Here's the drawing with two shaded views (mm, measured from the low corner). I have some questions. A direction names the side the tool comes from. Round coordinates to 2 decimals unless told otherwise and drop trailing zeros. Loops run counter-clockwise (first coordinate to the right, second up) from the corner with the lowest first, then second, coordinate; pieces in that order, holes last.
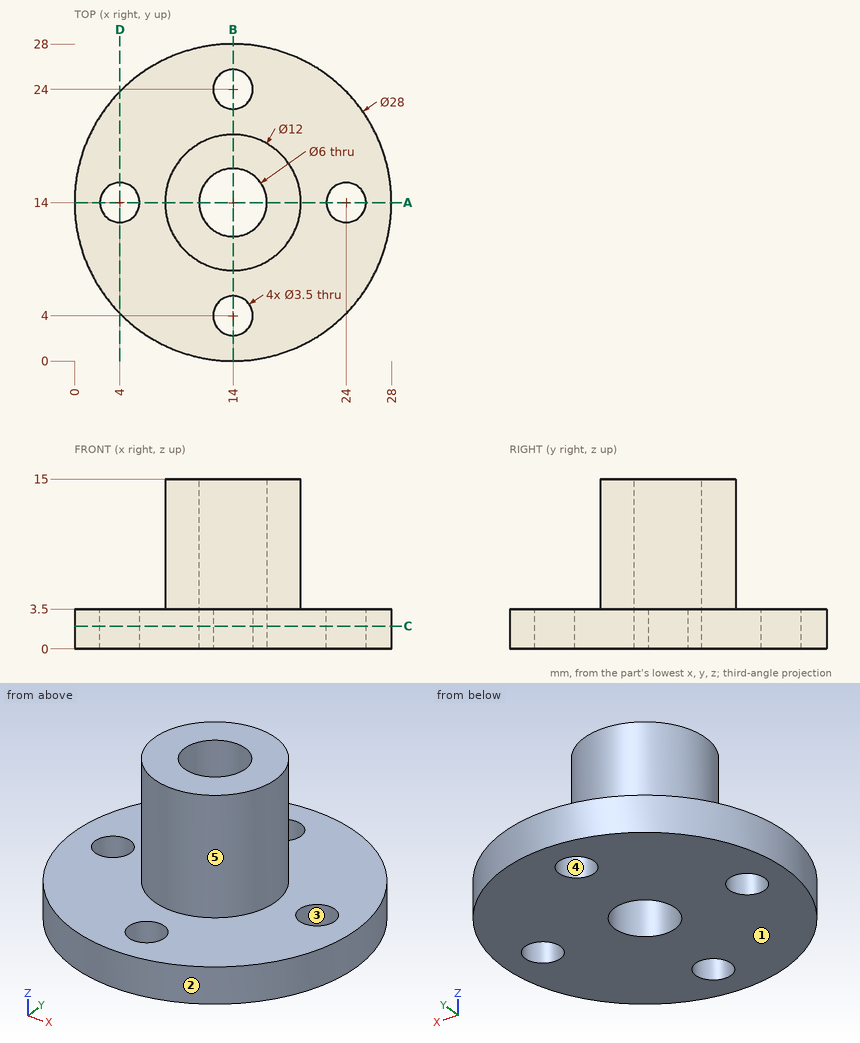
Item 1: Will these pins go through, and if not, where does the flat tip stop? pin 1 (5.5 mm diameter, centred on x = 14, y = 24, fed in from +Z); pin 2 (5 mm diameter, centred on x = 9.5, z = 5.5, fed in from -Y); pin 3 (1.5 mm diameter, centred on x = 11.5, z = 12.5, fed in from -Y).
Results list:
pin 1: stops at z = 3.5
pin 2: stops at y = 0.33
pin 3: stops at y = 8.26
Item 2: If we section it at A-A, the plane y = 14: Please give me the cut outline in (x, z).
Results list:
outline: (0, 0) - (2.25, 0) - (2.25, 3.5) - (0, 3.5) - close; (5.75, 0) - (11, 0) - (11, 15) - (8, 15) - (8, 3.5) - (5.75, 3.5) - close; (17, 0) - (22.25, 0) - (22.25, 3.5) - (20, 3.5) - (20, 15) - (17, 15) - close; (25.75, 0) - (28, 0) - (28, 3.5) - (25.75, 3.5) - close
Item 3: If I drill on line 1 along Y through (x, z) = (14, 2.7); line 2 along Y through (x, z) = (14, 11.25); line 3 along Z through (x, y) = (6, 22.75), over which ranges is the centre line in solid material (lowest first)?
Results list:
line 1: y = 0 to 2.25, 5.75 to 11, 17 to 22.25, 25.75 to 28
line 2: y = 8 to 11, 17 to 20
line 3: z = 0 to 3.5
Item 4: We'd pull the mould along X, two halves only. Please class the marked faces 1, 2 and 3: released by +X, released by -X, zero draft, split by the parting line, or undercut.
Results list:
face 1: zero draft
face 2: split by the parting line
face 3: undercut
Item 5: For the marked faces 4 and 5, which set-ups out of +Z, -Z, +X, -X, +Y, -Y let a thin tool reach every point of the face, with its end or its side?
Results list:
face 4: +Z, -Z
face 5: +Z
Item 6: If we section it at D-D, the plane x = 4: Please give me the cut outline in (y, z).
Results list:
outline: (4.2, 0) - (12.25, 0) - (12.25, 3.5) - (4.2, 3.5) - close; (15.75, 0) - (23.8, 0) - (23.8, 3.5) - (15.75, 3.5) - close
Item 7: If we section it at C-C, the plane z = 2: Please give me the cut outline in (x, y).
Results list:
outline: circle Ø28 at (14, 14); hole circle Ø3.5 at (4, 14); hole circle Ø6 at (14, 14); hole circle Ø3.5 at (14, 4); hole circle Ø3.5 at (14, 24); hole circle Ø3.5 at (24, 14)
